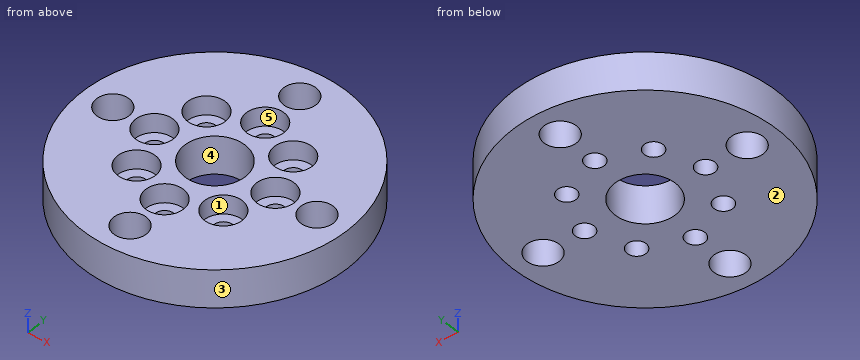
from build123d import *

# Parameters (mm, degrees)
DISC_PROFILE_70_R                  = 35
DISC_70_X_10_DEPTH                 = 10
CENTRE_BORE_PROFILE_16_R           = 8
CENTRE_BORE_16_DEPTH               = 10
OUTER_HOLES_PROFILE_4X_8_6_R       = 4.3
OUTER_HOLES_4X_8_6_DEPTH           = 10
COUNTERBORE_PROFILE_R              = 5
COUNTERBORES_DEPTH_5_DEPTH         = 5
COUNTERBORE_THROUGH_HOLE_PROFILE_R = 2.5
COUNTERBORE_THROUGH_HOLES_DEPTH    = 5


with BuildPart() as part:
    # Disc Profile Ø70 → Disc Ø70 x 10 (new body)
    with BuildSketch(Plane.XY):
        Circle(DISC_PROFILE_70_R)
    extrude(amount=DISC_70_X_10_DEPTH)

    # Centre Bore Profile Ø16 → Centre Bore Ø16 (cut)
    with BuildSketch(Plane.XY.offset(10)):
        Circle(CENTRE_BORE_PROFILE_16_R)
    extrude(amount=-CENTRE_BORE_16_DEPTH, mode=Mode.SUBTRACT)

    # Outer Holes Profile 4xØ8.6 → Outer Holes 4xØ8.6 (cut)
    with BuildSketch(Plane.XY.offset(10)):
        with Locations((0, 27)):
            Circle(OUTER_HOLES_PROFILE_4X_8_6_R)
        with Locations((27, 0)):
            Circle(OUTER_HOLES_PROFILE_4X_8_6_R)
        with Locations((0, -27)):
            Circle(OUTER_HOLES_PROFILE_4X_8_6_R)
        with Locations((-27, 0)):
            Circle(OUTER_HOLES_PROFILE_4X_8_6_R)
    extrude(amount=-OUTER_HOLES_4X_8_6_DEPTH, mode=Mode.SUBTRACT)

    # Counterbore Profile → Counterbores Depth 5 (cut)
    with BuildSketch(Plane.XY.offset(10)):
        with Locations((0, 16)):
            Circle(COUNTERBORE_PROFILE_R)
        with Locations((16, 0)):
            Circle(COUNTERBORE_PROFILE_R)
        with Locations((0, -16)):
            Circle(COUNTERBORE_PROFILE_R)
        with Locations((-16, 0)):
            Circle(COUNTERBORE_PROFILE_R)
        with Locations((11.492535714, -11.132008932)):
            Circle(COUNTERBORE_PROFILE_R)
        with Locations((11.313708499, 11.313708499)):
            Circle(COUNTERBORE_PROFILE_R)
        with Locations((-11.492535714, 11.132008932)):
            Circle(COUNTERBORE_PROFILE_R)
        with Locations((-11.313708499, -11.313708499)):
            Circle(COUNTERBORE_PROFILE_R)
    extrude(amount=-COUNTERBORES_DEPTH_5_DEPTH, mode=Mode.SUBTRACT)

    # Counterbore Through Hole Profile → Counterbore Through Holes (cut)
    with BuildSketch(Plane.XY.offset(5)):
        with Locations((0, 16)):
            Circle(COUNTERBORE_THROUGH_HOLE_PROFILE_R)
        with Locations((11.313708499, 11.313708499)):
            Circle(COUNTERBORE_THROUGH_HOLE_PROFILE_R)
        with Locations((16, 0)):
            Circle(COUNTERBORE_THROUGH_HOLE_PROFILE_R)
        with Locations((11.492535714, -11.132008932)):
            Circle(COUNTERBORE_THROUGH_HOLE_PROFILE_R)
        with Locations((0, -16)):
            Circle(COUNTERBORE_THROUGH_HOLE_PROFILE_R)
        with Locations((-11.313708499, -11.313708499)):
            Circle(COUNTERBORE_THROUGH_HOLE_PROFILE_R)
        with Locations((-16, 0)):
            Circle(COUNTERBORE_THROUGH_HOLE_PROFILE_R)
        with Locations((-11.492535714, 11.132008932)):
            Circle(COUNTERBORE_THROUGH_HOLE_PROFILE_R)
    extrude(amount=-COUNTERBORE_THROUGH_HOLES_DEPTH, mode=Mode.SUBTRACT)


solid = part.part
The model under review builds one solid part; all positions refer to its coordinate system, in mm. Face numbers are marked on the shaded views. A direction names the side the tool comes from. Round coordinates to 2 decimals unless told otherwise and drop trailing zeros. Loops run counter-clockwise (first coordinate to the right, second up) from the corner with the lowest first, then second, coordinate; pieces in that order, holes last. Notation, with made-up numbers: (39.25, -11.5) -> (54.25, -11.5) arc R33 cw to (54.25, 25.5) -> close; hole circle Ø6 at (56, 85.5). An arc over 180 degrees is marked (long way). Answer as CSV lines item,"result".
1) Add section B-B on x = -25. Write out the cut boundary in (y, z).
Geometry results:
outline,"(-24.49, 0) -> (-3.81, 0) -> (-3.81, 10) -> (-24.49, 10) -> close; (3.81, 0) -> (24.49, 0) -> (24.49, 10) -> (3.81, 10) -> close"
2) Add section A-A on y = -27. Write out the cut boundary in (x, z).
Geometry results:
outline,"(-22.27, 0) -> (-4.3, 0) -> (-4.3, 10) -> (-22.27, 10) -> close; (4.3, 0) -> (22.27, 0) -> (22.27, 10) -> (4.3, 10) -> close"
3) Add section C-C on z = 2.75. State how many separate pieces and enclosed holes the cut face has, plus the area to 3 significant figures.
Geometry results:
separate pieces,"1"
enclosed holes,"13"
area,"3,260 mm²"
4) To check wall thickness, follow line 1 along X through (y, z) = (10, 4.5); line 2 along X through (y, z) = (-12.5, 7.5); line 3 along X through (y, z) = (-8.5, 5.75). State the ranges of each line that lie inside material, in increasing order. Write a range as from..to.
Geometry results:
line 1,"x = -33.54..-13.72, -9.26..9.19, 13.44..33.54"
line 2,"x = -32.69..-16.17, -6.46..-3.57, 3.57..6.68, 16.3..32.69"
line 3,"x = -33.95..-15.45, -7.18..7.24, 15.74..33.95"
5) Tool access review of the marked faces 4 and 5: name each direction out of +Z, -Z, +X, -X, +Y, -Y from which nothing blocks a thin tool from reaching the whole face with its end or side.
Geometry results:
face 4,"+Z, -Z"
face 5,"+Z"
6) For P1, Ø11.5, axis at x = -16, y = 0, coming from the -Z side; P2, Ø5, axis at x = 16.5, y = -1, coming from the +Z side; P3, Ø3, axis at x = -0.5, z = 4.5, coming from the -Y side, all flat-tipped, find the tip position at first contact; note any pin that passes through.
Geometry results:
P1,"stops at z = 0"
P2,"stops at z = 5"
P3,"stops at y = -35"
7) Draft analysis for pull direction X (two halves, no side actions). For the marked faces 1, 2 and 3, state which applies: pulls with the +X half, pulls with the -X half, needs draft (parallel to the pull), parting line crosses it, or undercut.
Geometry results:
face 1,"undercut"
face 2,"needs draft"
face 3,"parting line crosses it"
